Could you check a few things on this model? Use its own coordinates, in mm. Face numbers are marked on the shaded views. A direction names the side the tool comes from. Round coordinates to 2 decimals unless told otherwise and drop trailing zeros. Write each loop counter-clockwise with the first axis right and the second up, starting at its lowest first coordinate (ties: lowest second). Pieces come first, ordered by that corner, then holes. Notation, with made-up numbers: (64.5, -20.75) -> (84.5, -20.75) arc R6 cw to (84.5, -9.75) -> close; hole circle Ø3 at (49, 15.25). An arc over 180 degrees is marked (long way). One line per question, with ' | ' between items. Start each with the question number.
1. For pin 1 Ø15 at (x, y) = (-10, 2) entering from +Z; pin 2 Ø5 at (x, y) = (-4.5, 3) entering from -Z; pin 3 Ø6 at (x, y) = (3, -11.5) entering from +Z, each with a flat end and sliding along its axis, tell me the tip position at first contact or that it passes through.
2. Thinking about a two-plate mould opening in X: for the marked faces 4, 5, 6 and 7, which applies, released by +X, released by -X, zero draft, split by the parting line, or undercut?
3. For the marked faces 1, 2 and 3, which set-ups out of +Z, -Z, +X, -X, +Y, -Y let a thin tool reach every point of the face, with its end or its side?
4. Imagine slicing it at D-D, the plane y = 10. List the corners of the cut face in (x, z) for me, and give its area (3 significant figures).
5. Imagine slicing it at A-A, the plane x = 24.8. List the corners of the cut face in (y, z) for me.
6. Imagine slicing it at C-C, the plane y = -20. List the corners of the cut face in (x, z) for me, and give its area (3 significant figures).
7. Imagine slicing it at B-B, the plane z = 9.25. List the corners of the cut face in (x, y) for me, and give its area (3 significant figures).
8. If I drill on line 1 along Y through (x, z) = (-4, 4.5); line 2 along X through (y, z) = (-10, 5.75); line 3 along X through (y, z) = (-20, 2.5), over which ranges is the centre line in solid material (lowest first)? Write a range as [from, to].
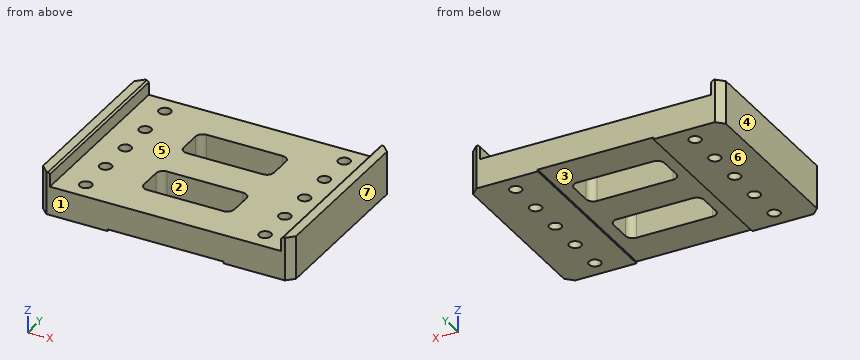
from build123d import *

# Parameters (mm, degrees)
SKETCH1_W           = 70
SKETCH1_H           = 50
BOSS_EXTRUDE1_DEPTH = 12
SKETCH2_W           = 64
SKETCH2_H           = 4
CUT_EXTRUDE1_DEPTH  = 63.20128616
CHAMFER1_SIZE       = 0.5
SKETCH3_W           = 32
SKETCH3_H           = 0.5
CUT_EXTRUDE2_DEPTH  = 63.20128616
LPATTERN1_COUNT     = 5
LPATTERN1_PITCH     = 10
SKETCH7_W           = 25
SKETCH7_H           = 10
CUT_EXTRUDE3_DEPTH  = 44.749285708
FILLET1_R           = 2
CHAMFER2_SIZE       = 2


with BuildPart() as part:
    # Sketch1 → Boss-Extrude1 (new body)
    with BuildSketch(Plane.XY):
        Rectangle(SKETCH1_W, SKETCH1_H)
    extrude(amount=BOSS_EXTRUDE1_DEPTH)

    # Sketch2 → Cut-Extrude1 (cut, through all)
    with BuildSketch(Plane.XZ.offset(25)):
        with Locations((0, 10)):
            Rectangle(SKETCH2_W, SKETCH2_H)
    extrude(amount=-CUT_EXTRUDE1_DEPTH, mode=Mode.SUBTRACT)

    # Chamfer1
    chamfer1_edges = [part.edges().sort_by_distance(p)[0] for p in [
        (-32, 0, 12),
        (32, 0, 12),
    ]]
    chamfer(chamfer1_edges, length=CHAMFER1_SIZE)

    # Sketch3 → Cut-Extrude2 (cut, through all)
    with BuildSketch(Plane(origin=(0, 25, 0), x_dir=(1, 0, 0), z_dir=(0, 1, 0))):
        with Locations((0, -0.25)):
            Rectangle(SKETCH3_W, SKETCH3_H)
    extrude(amount=-CUT_EXTRUDE2_DEPTH, mode=Mode.SUBTRACT)

    # Sketch6 → M4 Tapped Hole1 (revolve, cut)
    with BuildSketch(Plane(origin=(-24.8, 20, 8), x_dir=(0, -1, 0), z_dir=(1, 0, 0))):
        Polygon((0, 0), (0, 12.491420021), (1.65, 11.5), (1.65, 0), align=None)
    m4_tapped_hole1 = revolve(axis=Axis((-24.8, 20, 14.35), (0, 0, -1)), mode=Mode.SUBTRACT)

    # LPattern1: M4 Tapped Hole1 ×5
    with Locations(*[(0, -i * LPATTERN1_PITCH, 0) for i in range(1, LPATTERN1_COUNT)]):
        add(m4_tapped_hole1, mode=Mode.SUBTRACT)

    # Mirror1: M4 Tapped Hole1 across plane
    add(m4_tapped_hole1.mirror(Plane(origin=(0, 0, 0), x_dir=(0, 0, 1), z_dir=(1, 0, 0))), mode=Mode.SUBTRACT)

    # Mirror1 copy 1 sketch → Mirror1 copy 1 (revolve, cut)
    with BuildSketch(Plane(origin=(24.8, 10, 8), x_dir=(0, -1, 0), z_dir=(-1, 0, 0))):
        Polygon((0, 0), (0, -12.491420021), (1.65, -11.5), (1.65, 0), align=None)
    revolve(axis=Axis((24.8, 10, 14.35), (0, 0, 1)), mode=Mode.SUBTRACT)

    # Mirror1 copy 2 sketch → Mirror1 copy 2 (revolve, cut)
    with BuildSketch(Plane(origin=(24.8, 0, 8), x_dir=(0, -1, 0), z_dir=(-1, 0, 0))):
        Polygon((0, 0), (0, -12.491420021), (1.65, -11.5), (1.65, 0), align=None)
    revolve(axis=Axis((24.8, 0, 14.35), (0, 0, 1)), mode=Mode.SUBTRACT)

    # Mirror1 copy 3 sketch → Mirror1 copy 3 (revolve, cut)
    with BuildSketch(Plane(origin=(24.8, -10, 8), x_dir=(0, -1, 0), z_dir=(-1, 0, 0))):
        Polygon((0, 0), (0, -12.491420021), (1.65, -11.5), (1.65, 0), align=None)
    revolve(axis=Axis((24.8, -10, 14.35), (0, 0, 1)), mode=Mode.SUBTRACT)

    # Mirror1 copy 4 sketch → Mirror1 copy 4 (revolve, cut)
    with BuildSketch(Plane(origin=(24.8, -20, 8), x_dir=(0, -1, 0), z_dir=(-1, 0, 0))):
        Polygon((0, 0), (0, -12.491420021), (1.65, -11.5), (1.65, 0), align=None)
    revolve(axis=Axis((24.8, -20, 14.35), (0, 0, 1)), mode=Mode.SUBTRACT)

    # Sketch7 → Cut-Extrude3 (cut, through all)
    with BuildSketch(Plane.XY.offset(8)):
        with Locations((0, -10)):
            Rectangle(SKETCH7_W, SKETCH7_H)
        with Locations((0, 10)):
            Rectangle(SKETCH7_W, SKETCH7_H)
    extrude(amount=-CUT_EXTRUDE3_DEPTH, mode=Mode.SUBTRACT)

    # Fillet1
    fillet1_edges = [part.edges().sort_by_distance(p)[0] for p in [
        (-12.5, -15, 4.25),
        (-12.5, -5, 4.25),
        (12.5, -5, 4.25),
        (12.5, -15, 4.25),
        (12.5, 5, 4.25),
        (-12.5, 5, 4.25),
        (-12.5, 15, 4.25),
        (12.5, 15, 4.25),
    ]]
    fillet(fillet1_edges, radius=FILLET1_R)

    # Chamfer2
    chamfer2_edges = [part.edges().sort_by_distance(p)[0] for p in [
        (35, -25, 6),
        (-35, -25, 6),
        (-35, 25, 6),
        (35, 25, 6),
    ]]
    chamfer(chamfer2_edges, length=CHAMFER2_SIZE)


solid = part.part
Geometry results:
1) pin 1: stops at z = 8 | pin 2: stops at z = 0.5 | pin 3: passes through
2) face 4: released by -X | face 5: undercut | face 6: zero draft | face 7: released by +X
3) face 1: +Z, -Z, +X, -X, -Y | face 2: +Z, -Z | face 3: -Z, +Y, -Y
4) outline: (-35, 0) -> (-26.45, 0) -> (-26.45, 8) -> (-32, 8) -> (-32, 11.5) -> (-32.5, 12) -> (-35, 12) -> close; (-23.15, 0) -> (-16, 0) -> (-16, 0.5) -> (-12.5, 0.5) -> (-12.5, 8) -> (-23.15, 8) -> close; (12.5, 0.5) -> (16, 0.5) -> (16, 0) -> (23.15, 0) -> (23.15, 8) -> (12.5, 8) -> close; (26.45, 0) -> (35, 0) -> (35, 12) -> (32.5, 12) -> (32, 11.5) -> (32, 8) -> (26.45, 8) -> close | area: 327 mm2
5) outline: (-25, 0) -> (-21.65, 0) -> (-21.65, 8) -> (-25, 8) -> close; (-18.35, 0) -> (-11.65, 0) -> (-11.65, 8) -> (-18.35, 8) -> close; (-8.35, 0) -> (-1.65, 0) -> (-1.65, 8) -> (-8.35, 8) -> close; (1.65, 0) -> (8.35, 0) -> (8.35, 8) -> (1.65, 8) -> close; (11.65, 0) -> (18.35, 0) -> (18.35, 8) -> (11.65, 8) -> close; (21.65, 0) -> (25, 0) -> (25, 8) -> (21.65, 8) -> close
6) outline: (-35, 0) -> (-26.45, 0) -> (-26.45, 8) -> (-32, 8) -> (-32, 11.5) -> (-32.5, 12) -> (-35, 12) -> close; (-23.15, 0) -> (-16, 0) -> (-16, 0.5) -> (16, 0.5) -> (16, 0) -> (23.15, 0) -> (23.15, 8) -> (-23.15, 8) -> close; (26.45, 0) -> (35, 0) -> (35, 12) -> (32.5, 12) -> (32, 11.5) -> (32, 8) -> (26.45, 8) -> close | area: 515 mm2
7) outline: (-35, -23) -> (-33, -25) -> (-32, -25) -> (-32, 25) -> (-33, 25) -> (-35, 23) -> close; (32, -25) -> (33, -25) -> (35, -23) -> (35, 23) -> (33, 25) -> (32, 25) -> close | area: 292 mm2
8) line 1: y = [-25, -15], [-5, 5], [15, 25] | line 2: x = [-35, -26.45], [-23.15, -12.5], [12.5, 23.15], [26.45, 35] | line 3: x = [-35, -26.45], [-23.15, 23.15], [26.45, 35]
